The drawing under review shows one solid part. Ordinate dimensions are in mm from its lowest x, y, z. Give positions to 0.01 mm unless a question says otherwise; leave off trailing zeros. Write each loop counter-clockwise with the first axis right and the second up, starting at its lowest first coordinate (ties: lowest second). Pieces come first, ordered by that corner, then holes.
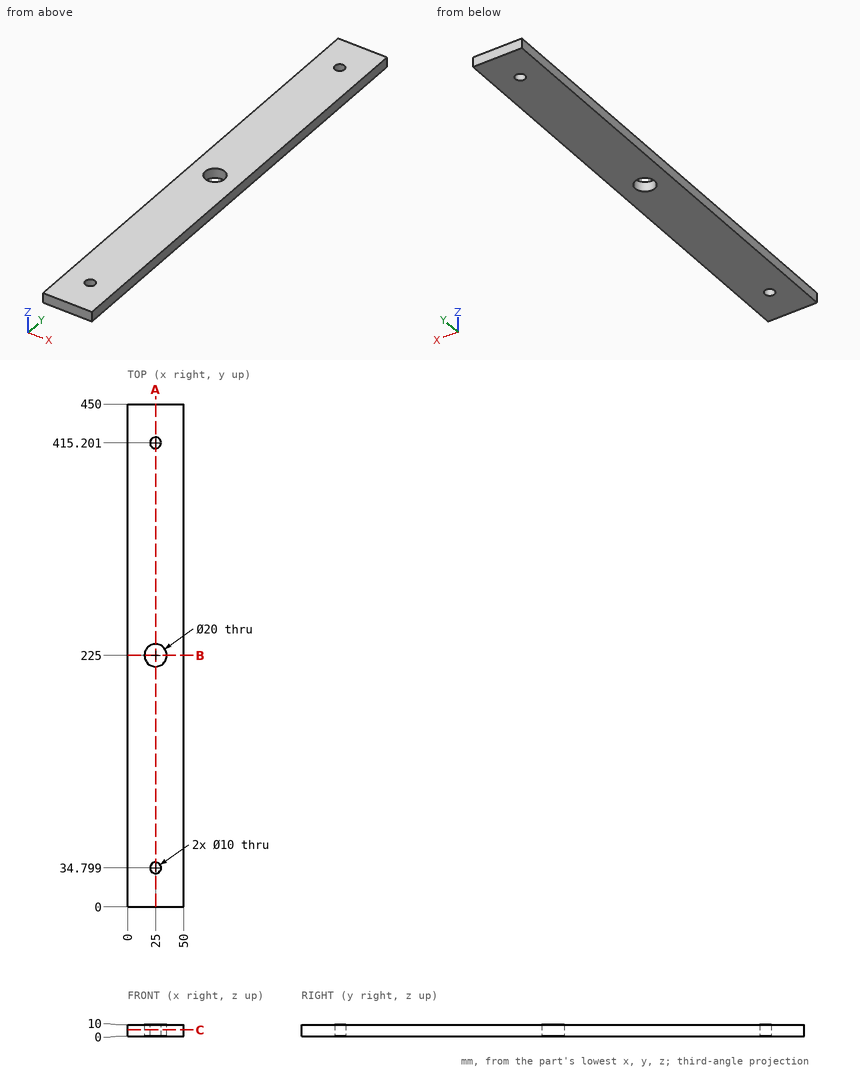
1) Consider section C-C, the plane z = 5.5. Give the boundary of the cut face in (x, y), then the cut area to 3 significant figures.
2) Consider section A-A, the plane x = 25. Give the boundary of the cut face in (y, z), then the cut area to 3 significant figures.
3) To check wall thickness, follow probe 1 along Y at (x, z) = (25, 2.75); probe 2 along Y at (x, z) = (23, 9.25); probe 3 along X at (y, z) = (32, 2.75). State the ranges of each line that lie inside material, in increasing order.
4) Insertion check: pin 1 (6 mm diameter, centred on x = 25, y = 34.8, fed in from +Z). The pin has a flat end and moves straight along its axis. Give the tip position at first contact, or say it passes through.
5) Consider section B-B, the plane y = 225. Give the boundary of the cut face in (x, z), then the cut area to 3 significant figures.
Answer block:
1. outline: (0, 0) - (50, 0) - (50, 450) - (0, 450) - close; hole circle Ø20 at (25, 225); hole circle Ø10 at (25, 34.8); hole circle Ø10 at (25, 415.2)
1. area: 22,000 mm2
2. outline: (0, 0) - (29.8, 0) - (29.8, 10) - (0, 10) - close; (39.8, 0) - (215, 0) - (215, 10) - (39.8, 10) - close; (235, 0) - (410.2, 0) - (410.2, 10) - (235, 10) - close; (420.2, 0) - (450, 0) - (450, 10) - (420.2, 10) - close
2. area: 4,100 mm2
3. probe 1: y = 0 to 29.8, 39.8 to 215, 235 to 410.2, 420.2 to 450
3. probe 2: y = 0 to 30.22, 39.38 to 215.2, 234.8 to 410.62, 419.78 to 450
3. probe 3: x = 0 to 20.86, 29.14 to 50
4. pin 1: passes through
5. outline: (0, 0) - (15, 0) - (15, 10) - (0, 10) - close; (35, 0) - (50, 0) - (50, 10) - (35, 10) - close
5. area: 300 mm2
